Read the model definition and answer for the solid it produces. Units are mm, in the model's axes. Round coordinates to 2 decimals unless told otherwise and drop trailing zeros. Loops run counter-clockwise (first coordinate to the right, second up) from the corner with the lowest first, then second, coordinate; pieces in that order, holes last. Notation, with made-up numbers: (82, -15) - (120, -15) arc R25 ccw to (120, 20) - close; hole circle Ø4 at (6.5, -15). An arc over 180 degrees is marked (long way). Use CSV: the item, a comma, the result in double quotes. Start each with the question number.
1. Find section D-D (x = -11). Give the vertices of the cut face in (y, z), and give its area (3 significant figures).
2. Find section C-C (z = 2.25). Give the vertices of the cut face in (x, y).
3. Consider line 1 along Y through (x, z) = (37, 1.35); line 2 along Y through (x, z) = (-19, 7.5); line 3 along Y through (x, z) = (34, 5). Determine where each line is inside the solid, lowest interval first.
4. Find section B-B (y = -117). Give the vertices of the cut face in (x, z), and give its area (4 significant figures).
5. Given pin 1 Ø3.5 at (x, y) = (37, -117) entering from +Z; pin 2 Ø14.5 at (x, y) = (-17, -10) entering from +Z; pin 3 Ø7 at (x, y) = (-17, -117) entering from +Z; pin 4 Ø3.5 at (x, y) = (33, -86) entering from -Z, each flat-ended and moving along its own axis, determine where each tip first touches the part or whether it passes through.
6. Find section A-A (x = 10). Give the vertices of the cut face in (y, z), and give its area (3 significant figures).
from build123d import *

# Parameters (mm, degrees)
SKETCH_1_W                  = 64
SKETCH_1_H                  = 130
EXTRUDE_1_DEPTH             = 10
HOLE_WIZARD_0_D             = 5.5
HOLE_WIZARD_0_CBORE_D       = 9
HOLE_WIZARD_0_CBORE_DEPTH   = 5.5
HOLE_WIZARD_C_1_D           = 6.5
HOLE_WIZARD_C_1_CBORE_D     = 12
HOLE_WIZARD_C_1_CBORE_DEPTH = 6.5
CHAMFER_1_SIZE              = 1


with BuildPart() as part:
    # 草图1 → 凸台-拉伸1 (new body)
    with BuildSketch(Plane.XY):
        with Locations((10, -65)):
            Rectangle(SKETCH_1_W, SKETCH_1_H)
    extrude(amount=EXTRUDE_1_DEPTH)

    # 打孔尺寸根据内六角圆柱头螺钉的类型0 (through all)
    with Locations(Plane.XY.offset(10)):
        with Locations((-17, -10), (37, -10), (-17, -117), (37, -117)):
            CounterBoreHole(HOLE_WIZARD_0_D / 2, HOLE_WIZARD_0_CBORE_D / 2, HOLE_WIZARD_0_CBORE_DEPTH)

    # 打孔尺寸根据六角头螺栓 C 级的类型1 (through all)
    with Locations(Plane(origin=(0, 0, 0), x_dir=(-1, 0, 0), z_dir=(0, 0, -1))):
        with Locations((10, -86.5), (-10, -86.5), (-30, -86.5)):
            CounterBoreHole(HOLE_WIZARD_C_1_D / 2, HOLE_WIZARD_C_1_CBORE_D / 2, HOLE_WIZARD_C_1_CBORE_DEPTH)

    # 倒角1
    chamfer_1_edges = [part.edges().sort_by_distance(p)[0] for p in [
        (-22, 0, 5),
        (42, 0, 5),
        (42, -130, 5),
        (-22, -130, 5),
    ]]
    chamfer(chamfer_1_edges, length=CHAMFER_1_SIZE)


solid = part.part
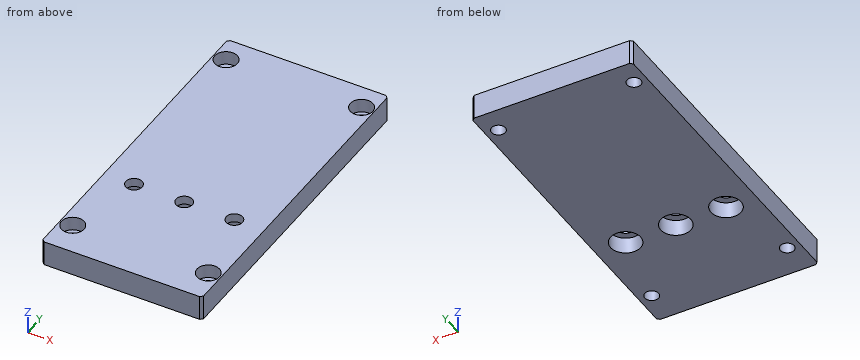
Filled sheet:
1,outline,"(-130, 0) - (-92.42, 0) - (-92.42, 6.5) - (-89.59, 6.5) - (-89.59, 10) - (-130, 10) - close; (-83.41, 6.5) - (-80.58, 6.5) - (-80.58, 0) - (0, 0) - (0, 10) - (-83.41, 10) - close"
1,area,"1,200 mm²"
2,outline,"(-22, -129) - (-21, -130) - (41, -130) - (42, -129) - (42, -1) - (41, 0) - (-21, 0) - (-22, -1) - close; hole circle Ø5.5 at (-17, -117); hole circle Ø5.5 at (-17, -10); hole circle Ø12 at (-10, -86.5); hole circle Ø12 at (10, -86.5); hole circle Ø12 at (30, -86.5); hole circle Ø5.5 at (37, -117); hole circle Ø5.5 at (37, -10)"
3,line 1,"y = -130 to -119.75, -114.25 to -12.75, -7.25 to 0"
3,line 2,"y = -130 to -121.03, -112.97 to -14.03, -5.97 to 0"
3,line 3,"y = -130 to -120.35, -113.65 to -90.97, -82.03 to -13.35, -6.65 to 0"
4,outline,"(-22, 0) - (-19.75, 0) - (-19.75, 4.5) - (-21.5, 4.5) - (-21.5, 10) - (-22, 10) - close; (-14.25, 0) - (34.25, 0) - (34.25, 4.5) - (32.5, 4.5) - (32.5, 10) - (-12.5, 10) - (-12.5, 4.5) - (-14.25, 4.5) - close; (39.75, 0) - (42, 0) - (42, 10) - (41.5, 10) - (41.5, 4.5) - (39.75, 4.5) - close"
4,area,"491.5 mm²"
5,pin 1,"passes through"
5,pin 2,"stops at z = 10"
5,pin 3,"stops at z = 4.5"
5,pin 4,"stops at z = 6.5"
6,outline,"(-130, 0) - (-92.5, 0) - (-92.5, 6.5) - (-89.75, 6.5) - (-89.75, 10) - (-130, 10) - close; (-83.25, 6.5) - (-80.5, 6.5) - (-80.5, 0) - (0, 0) - (0, 10) - (-83.25, 10) - close"
6,area,"1,200 mm²"
